Check sheet for the modelled part. Datum: model origin and axes. Units: mm. Face numbers are marked on the shaded views. Coordinates: 2 decimals unless noted, no trailing zeros. Order: outer loops, then holes, each group sorted by start corner. A loop starts at its lowest first (then second) coordinate and runs counter-clockwise, first axis right, second up.
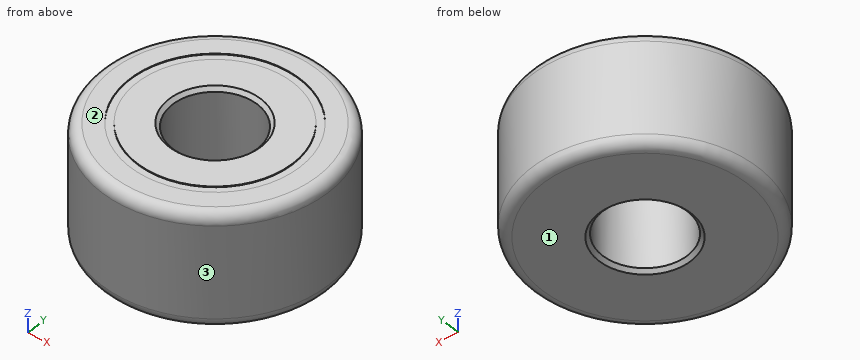
from build123d import *

# Parameters (mm, degrees)
SKETCH1_R           = 16
BOSS_EXTRUDE1_DEPTH = 16
SKETCH2_R           = 6
CUT_EXTRUDE1_DEPTH  = 16
SKETCH3_R           = 12
SKETCH3_R_2         = 11
CUT_EXTRUDE2_DEPTH  = 0.1
FILLET1_R           = 1.5
CHAMFER1_SIZE       = 0.5


with BuildPart() as part:
    # Sketch1 → Boss-Extrude1 (new body)
    with BuildSketch(Plane.XY):
        Circle(SKETCH1_R)
    extrude(amount=BOSS_EXTRUDE1_DEPTH)

    # Sketch2 → Cut-Extrude1 (cut)
    with BuildSketch(Plane.XY.offset(16)):
        Circle(SKETCH2_R)
    extrude(amount=-CUT_EXTRUDE1_DEPTH, mode=Mode.SUBTRACT)

    # Sketch3 → Cut-Extrude2 (cut)
    with BuildSketch(Plane.XY.offset(16)):
        Circle(SKETCH3_R)
        Circle(SKETCH3_R_2, mode=Mode.SUBTRACT)
    extrude(amount=-CUT_EXTRUDE2_DEPTH, mode=Mode.SUBTRACT)

    # Fillet1
    fillet1_edges = [part.edges().sort_by_distance(p)[0] for p in [
        (-16, 0, 0),
        (-16, 0, 16),
    ]]
    fillet(fillet1_edges, radius=FILLET1_R)

    # Chamfer1
    chamfer1_edges = [part.edges().sort_by_distance(p)[0] for p in [
        (-6, 0, 0),
        (-6, 0, 16),
    ]]
    chamfer(chamfer1_edges, length=CHAMFER1_SIZE)


solid = part.part
(1) Cross-section at C-C (z = 3.75). Enter the section's corners in (x, y), and give its area (3 significant figures).
Filled in:
outline: circle Ø32 at (0, 0); hole circle Ø12 at (0, 0)
area: 691 mm2
(2) Cross-section at A-A (y = 0). Enter the section's corners in (x, z).
Filled in:
outline: (-16, 1.5) arc R1.5 ccw to (-14.5, 0) - (-6.5, 0) - (-6, 0.5) - (-6, 15.5) - (-6.5, 16) - (-11, 16) - (-11, 15.9) - (-12, 15.9) - (-12, 16) - (-14.5, 16) arc R1.5 ccw to (-16, 14.5) - close; (6, 0.5) - (6.5, 0) - (14.5, 0) arc R1.5 ccw to (16, 1.5) - (16, 14.5) arc R1.5 ccw to (14.5, 16) - (12, 16) - (12, 15.9) - (11, 15.9) - (11, 16) - (6.5, 16) - (6, 15.5) - close
(3) Release check for a two-part mould opening along Z. For the marked faces 1, 2 and 3 record: +Z half, -Z half, draft (parallel to the pull), parting line (faces both ways), or undercut.
Filled in:
face 1: -Z half
face 2: +Z half
face 3: draft
(4) Thickness scan on probe 1 along Y at (x, z) = (0, 4.5); probe 2 along Y at (x, z) = (-5, 10); probe 3 along X at (y, z) = (-4.5, 6). Record the ranges inside material, lowest first.
Filled in:
probe 1: y = -16 to -6, 6 to 16
probe 2: y = -15.2 to -3.32, 3.32 to 15.2
probe 3: x = -15.35 to -3.97, 3.97 to 15.35
(5) Go/stop test with flat-tipped pins: P1, Ø8, axis at x = -1.5, y = -6.5, coming from the -Z side; P2, Ø4, axis at x = -10, z = 7, coming from the +Y side; P3, Ø5, axis at y = 5, z = 9, coming from the +X side; P4, Ø4, axis at x = 12.5, z = 7, coming from the +Y side. Record where each tip stops, or that it passes through.
Filled in:
P1: stops at z = 0
P2: stops at y = 13.86
P3: stops at x = 15.8
P4: stops at y = 12.07
